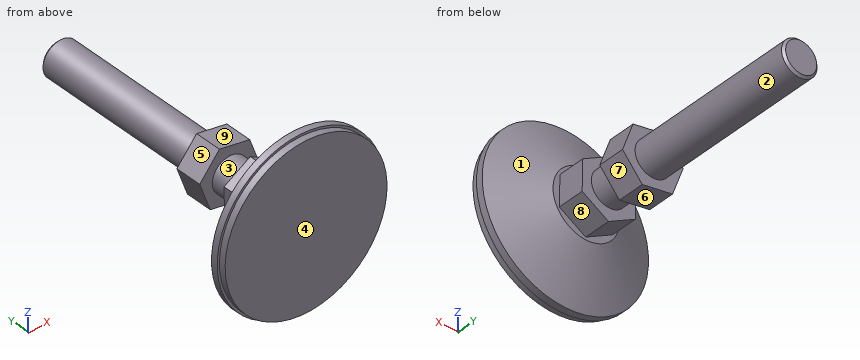
```python
from build123d import *

# Parameters (mm, degrees)
EXTRUDE1_DEPTH = 12
EXTRUDE2_START = 35
EXTRUDE2_DEPTH = 12
CHAMFER1_SIZE  = 1


with BuildPart() as part:
    # Sketch1 → Revolve1 (revolve)
    with BuildSketch(Plane.XY, mode=Mode.PRIVATE) as revolve1_sk:
        Polygon((-37.5, 10.372678427), (-15, 21.372678427), (-8, 21.372678427), (-8, 134.372678427), (0, 134.372678427), (0, 4.372678427), (-36.5, 4.372678427), (-36.5, 7.372678427), (-37.5, 7.372678427), align=None)
    revolve(revolve1_sk.sketch.rotate(Axis((0, 0, 0), (0, -1, 0)), 270), axis=Axis((0, 0, 0), (0, -1, 0)))

    # Sketch2 → Extrude1 (add)
    with BuildSketch(Plane(origin=(0, 21.372678427, 0), x_dir=(-1, 0, 0), z_dir=(0, 1, 0))):
        Polygon((-11.859328821, 7.166332389), (-12.135890312, -6.687313836), (-0.27656149, -13.853646226), (11.859328821, -7.166332389), (12.135890312, 6.687313836), (0.27656149, 13.853646226), align=None)
    extrude(amount=EXTRUDE1_DEPTH)

    # Sketch3 → Extrude2 (add)
    with BuildSketch(Plane(origin=(0, 21.372678427, 0), x_dir=(-1, 0, 0), z_dir=(0, 1, 0)).offset(EXTRUDE2_START)):
        Polygon((-8.887785091, 10.63048805), (-13.650165251, -2.381803647), (-4.76238016, -13.012291697), (8.887785091, -10.63048805), (13.650165251, 2.381803647), (4.76238016, 13.012291697), align=None)
    extrude(amount=-EXTRUDE2_DEPTH)

    # Chamfer1
    chamfer1_edges = [part.edges().sort_by_distance(p)[0] for p in [
        (0, 134.372678427, -8),
    ]]
    chamfer(chamfer1_edges, length=CHAMFER1_SIZE)


solid = part.part
```
Read the model definition and answer for the solid it produces. Units are mm, in the model's axes. Face numbers are marked on the shaded views. A direction names the side the tool comes from. Give positions to 0.01 mm unless a question says otherwise; leave off trailing zeros. Write each loop counter-clockwise with the first axis right and the second up, starting at its lowest first coordinate (ties: lowest second). Pieces come first, ordered by that corner, then holes. Notation, with made-up numbers: (60, 70.5) -> (70, 70.5) arc R8 ccw to (70, 84.5) -> close; hole circle Ø7 at (36, 20.25). An arc over 180 degrees is marked (long way). Answer in a Markdown table with one row per item.
1) Straight lines are drawn through the part: line 1 (Y direction, x = 11.5, z = 0); line 2 (Y direction, x = -27.5, z = 21); line 3 (Y direction, x = 23, z = -22). For each, find the intervals that lie inside material, in ascending order. Write a range as [from, to].
Results list:
| item | result |
|---|---|
| line 1 | [4.37, 33.37], [44.37, 56.37] |
| line 2 | [4.37, 11.79] |
| line 3 | [4.37, 13.15] |
2) Section C-C on y = 104 is taken. Give the vertices of the cut face in (x, z), plus the area to 3 significant figures.
Results list:
| item | result |
|---|---|
| outline | circle Ø16 at (0, 0) |
| area | 201 mm^2 |
3) A tool of negligible diameter and unlimited length cuts with its end or side. For the marked faces 5, 6, 7, 8 and 9, from which of +Z, -Z, +X, -X, +Y, -Y can it reach the whole face along a straight path? Write none if from no direction.
Results list:
| item | result |
|---|---|
| face 5 | +Z, -X, +Y |
| face 6 | -Z, -X, +Y |
| face 7 | -Z, +X, +Y |
| face 8 | -Z, +X |
| face 9 | +Z, +X, +Y |
4) Determine the mould class of the marked faces 1, 2, 3 and 4 for opening direction Y: released by +Y, released by -Y, zero draft, split by the parting line, or undercut.
Results list:
| item | result |
|---|---|
| face 1 | released by +Y |
| face 2 | zero draft |
| face 3 | undercut |
| face 4 | released by -Y |
5) Section B-B on z = 0 is taken. Give the vertices of the cut face in (x, y), plus the area to 3 significant figures.
Results list:
| item | result |
|---|---|
| outline | (-37.5, 7.37) -> (-36.5, 7.37) -> (-36.5, 4.37) -> (36.5, 4.37) -> (36.5, 7.37) -> (37.5, 7.37) -> (37.5, 10.37) -> (15, 21.37) -> (12, 21.37) -> (12, 33.37) -> (8, 33.37) -> (8, 44.37) -> (12.78, 44.37) -> (12.78, 56.37) -> (8, 56.37) -> (8, 133.37) -> (7, 134.37) -> (-7, 134.37) -> (-8, 133.37) -> (-8, 56.37) -> (-12.78, 56.37) -> (-12.78, 44.37) -> (-8, 44.37) -> (-8, 33.37) -> (-12, 33.37) -> (-12, 21.37) -> (-15, 21.37) -> (-37.5, 10.37) -> close |
| area | 3,040 mm^2 |
6) Section A-A on y = 53 is taken. Give the vertices of the cut face in (x, z), plus the area to 3 significant figures.
Results list:
| item | result |
|---|---|
| outline | (-13.65, 2.38) -> (-8.89, -10.63) -> (4.76, -13.01) -> (13.65, -2.38) -> (8.89, 10.63) -> (-4.76, 13.01) -> close |
| area | 499 mm^2 |
7) Each of these flat-tipped pins is pushed along its axis until it touches: pin 1 Ø10 at (x, y) = (-22.5, 55.5) entering from +Z; pin 2 Ø6 at (y, z) = (79.5, 3) entering from +X; pin 3 Ø3 at (x, z) = (5.5, 14.5) entering from +Y; pin 4 Ø1.5 at (x, y) = (8, 36) entering from +Z. Where does it stop, or does it pass through?
Results list:
| item | result |
|---|---|
| pin 1 | through |
| pin 2 | x = 8 |
| pin 3 | y = 21.37 |
| pin 4 | z = 3.38 |
